Can you work these out from the model? Positions are in its coordinate system, mm. Face numbers are marked on the shaded views. Give positions to 0.01 mm unless a question says otherwise; leave off trailing zeros. Order: outer loops, then holes, each group sorted by start corner. A loop starts at its lowest first (then second) coordinate and runs counter-clockwise, first axis right, second up. Notation, with made-up numbers: (-9, -6.75) - (38, -6.75) arc R33 cw to (38, 31.25) - close; hole circle Ø4 at (33, 47.5). An arc over 180 degrees is marked (long way). Answer as a JSON object with one key per item and string values.
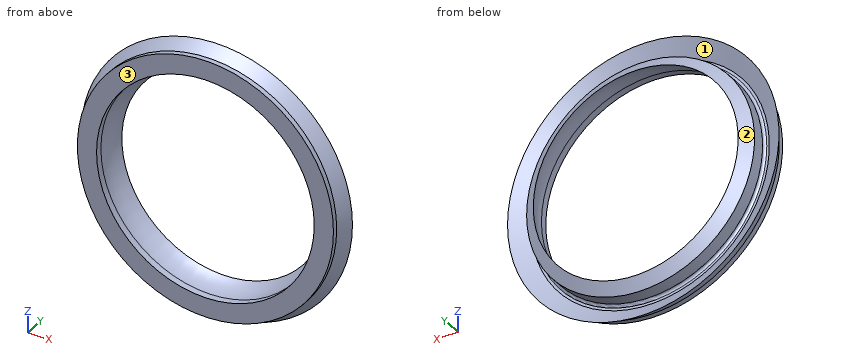
```python
from build123d import *


with BuildPart() as part:
    # 草图1 → 旋转1 (revolve)
    with BuildSketch(Plane.XY):
        with BuildLine():
            Line((42.5, -6.169872981), (49.995512501, -6.169872981))
            Line((49.995512501, -6.169872981), (49.995512501, -4.169872981))
            Line((49.995512501, -4.169872981), (53, 0.830127019))
            Line((53, 0.830127019), (46.5, -3.5))
            Line((46.5, -3.5), (45.5, -3.5))
            ThreePointArc((45.5, -3.5), (44.792893219, -3.207106781), (44.5, -2.5))
            Line((44.5, -2.5), (44.5, 2.5))
            Line((44.5, 2.5), (40, 5.5))
            ThreePointArc((40, 5.5), (41.968412898, 1.199559138), (42.5, -3.5))
            Line((42.5, -3.5), (42.5, -6.169872981))
        make_face()
    revolve(axis=Axis((0, -5.5, 0), (0, 1, 0)))


solid = part.part
```
Q1. We'd pull the mould along X, two halves only. Please class the marked faces 1, 2 and 3: released by +X, released by -X, zero draft, split by the parting line, or undercut.
Recorded:
{"face 1": "undercut", "face 2": "split by the parting line", "face 3": "zero draft"}
Q2. If we section it at A-A, the plane x = 0: Please give me the cut outline in (y, z).
Recorded:
{"outline": "(-6.17, -50) - (-4.17, -50) - (0.83, -53) - (-3.5, -46.5) - (-3.5, -45.5) arc R1 cw to (-2.5, -44.5) - (2.5, -44.5) - (5.5, -40) arc R15 cw to (-3.5, -42.5) - (-6.17, -42.5) - close; (-6.17, 42.5) - (-3.5, 42.5) arc R15 cw to (5.5, 40) - (2.5, 44.5) - (-2.5, 44.5) arc R1 cw to (-3.5, 45.5) - (-3.5, 46.5) - (0.83, 53) - (-4.17, 50) - (-6.17, 50) - close"}
Q3. If we section it at B-B, the plane z = 0: Please give me the cut outline in (x, y), then the cut area to 3 significant figures.
Recorded:
{"outline": "(-53, 0.83) - (-50, -4.17) - (-50, -6.17) - (-42.5, -6.17) - (-42.5, -3.5) arc R15 cw to (-40, 5.5) - (-44.5, 2.5) - (-44.5, -2.5) arc R1 cw to (-45.5, -3.5) - (-46.5, -3.5) - close; (40, 5.5) arc R15 cw to (42.5, -3.5) - (42.5, -6.17) - (50, -6.17) - (50, -4.17) - (53, 0.83) - (46.5, -3.5) - (45.5, -3.5) arc R1 cw to (44.5, -2.5) - (44.5, 2.5) - close", "area": "93.3 mm^2"}
Q4. I need wall thicknesses on L1, parallel to Z at x = 0, y = -4.6; L2, parallel to X at y = -3.25, z = -35. Which ranges of each line are inside material? Lowest first, please.
Recorded:
{"L1": "z = -50 to -42.5, 42.5 to 50", "L2": "x = -36.47 to -31.18, -28.03 to -24.13, 24.13 to 28.03, 31.18 to 36.47"}
Q5. I'm going to push flat-ended pins straight in: pin 1 Ø6 at (x, y) = (26.5, -0.5) entering from -Z; pin 2 Ø1.5 at (x, y) = (4.5, -1.5) entering from +Z; pin 3 Ø1.5 at (x, z) = (-24.5, -32) entering from -Y. Where does each tip first touch, or does it pass through?
Recorded:
{"pin 1": "stops at z = -47.35", "pin 2": "stops at z = 51.86", "pin 3": "stops at y = 3.65"}
